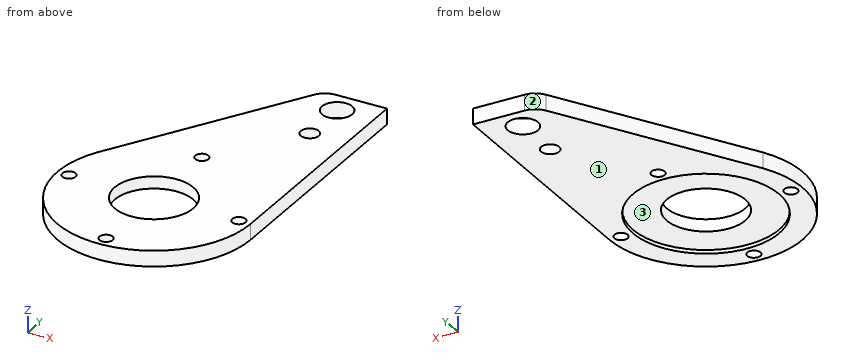
from build123d import *

# Parameters (mm, degrees)
SKETCH_1_R          = 32.5
SKETCH_1_R_2        = 12.5
SKETCH_1_R_3        = 7.5
EXTRUDE_1_DEPTH     = 13
CUT_EXTRUDE_START   = 3
SKETCH_2_R          = 60.5
CUT_EXTRUDE_2_DEPTH = 219.79851714
SKETCH_4_R          = 5.5
CUT_EXTRUDE_3_DEPTH = 216.79851714


with BuildPart() as part:
    # 草图1 → 凸台-拉伸1 (new body)
    with BuildSketch(Plane.XY):
        with BuildLine():
            Line((80, 200), (37.5, 200))
            ThreePointArc((37.5, 200), (29.674290769, 197.955582218), (23.848458927, 192.34478438))
            Line((23.848458927, 192.34478438), (-69.388730207, 39.814621941))
            ThreePointArc((-69.388730207, 39.814621941), (-20.602203565, -77.30167662), (80, 0))
            Line((80, 0), (80, 160))
            Line((80, 160), (80, 200))
        make_face()
        with Locations(Location((0, 0, 0), (0, 0, 180))):
            Circle(SKETCH_1_R, mode=Mode.SUBTRACT)
        with Locations(Location((50, 180, 0), (0, 0, 180))):
            Circle(SKETCH_1_R_2, mode=Mode.SUBTRACT)
        with Locations(Location((50, 140, 0), (0, 0, 180))):
            Circle(SKETCH_1_R_3, mode=Mode.SUBTRACT)
    extrude(amount=EXTRUDE_1_DEPTH)

    # 草图2 → 切除-拉伸2 (cut, through all)
    with BuildSketch(Plane.XY.offset(CUT_EXTRUDE_START)):
        Circle(SKETCH_2_R)
    extrude(amount=-CUT_EXTRUDE_2_DEPTH, mode=Mode.SUBTRACT)

    # 草图4 → 切除-拉伸3 (cut, through all)
    with BuildSketch(Plane(origin=(0, 0, 0), x_dir=(-1, 0, 0), z_dir=(0, 0, -1))):
        with Locations((70.25, 0)):
            Circle(SKETCH_4_R)
        with Locations((0, -70.25)):
            Circle(SKETCH_4_R)
        with Locations((-70.25, 0)):
            Circle(SKETCH_4_R)
        with Locations((0, 70.25)):
            Circle(SKETCH_4_R)
    extrude(amount=-CUT_EXTRUDE_3_DEPTH, mode=Mode.SUBTRACT)


solid = part.part
Work out the finished part from the listing and answer in its coordinate system (mm). Face numbers are marked on the shaded views. Round coordinates to 2 decimals unless told otherwise and drop trailing zeros. Write each loop counter-clockwise with the first axis right and the second up, starting at its lowest first coordinate (ties: lowest second). Pieces come first, ordered by that corner, then holes. Notation, with made-up numbers: M 65.5,-6.5 L 120.5,-6.5 A16 ccw 120.5,23.5 Z; hole C 29,27.5 d7. An arc over 180 degrees is marked long. Use a Markdown table: item, result.
1) The part is cut by section A-A on y = -70.25. Give the vertices of the cut face in (x, z), plus the area to 3 significant figures.
Taken from the geometry:
| item | result |
|---|---|
| outline | M -38.27,0 L -5.5,0 L -5.5,13 L -38.27,13 Z; M 5.5,0 L 38.27,0 L 38.27,13 L 5.5,13 Z |
| area | 852 mm2 |
2) Determine the mould class of the marked faces 1, 2 and 3 for opening direction Y: pulls with the +Y half, pulls with the -Y half, needs draft (parallel to the pull), parting line crosses it, or undercut.
Taken from the geometry:
| item | result |
|---|---|
| face 1 | needs draft |
| face 2 | pulls with the +Y half |
| face 3 | undercut |
3) Flat-ended cylindrical pins translate along their axes: pin 1 (1.5 mm diameter, centred on x = 9, z = 7.5, fed in from -Y); pin 2 (2 mm diameter, centred on x = -19, z = 1.5, fed in from -Y); pin 3 (1 mm diameter, centred on y = 160, z = 10, fed in from -X). Find the tip coordinate at first contact, or state that the pin passes through.
Taken from the geometry:
| item | result |
|---|---|
| pin 1 | stops at y = -79.57 |
| pin 2 | stops at y = -77.95 |
| pin 3 | stops at x = 3.77 |
4) The part is cut by section B-B on x = 54. Give the vertices of the cut face in (y, z).
Taken from the geometry:
| item | result |
|---|---|
| outline | M -59.03,0 L -27.28,0 L -27.28,3 L 27.28,3 L 27.28,0 L 133.66,0 L 133.66,13 L -59.03,13 Z; M 146.34,0 L 168.16,0 L 168.16,13 L 146.34,13 Z; M 191.84,0 L 200,0 L 200,13 L 191.84,13 Z |
5) The part is cut by section D-D on x = 17.5. Give the vertices of the cut face in (y, z).
Taken from the geometry:
| item | result |
|---|---|
| outline | M -78.06,0 L -57.91,0 L -57.91,3 L -27.39,3 L -27.39,13 L -78.06,13 Z; M 27.39,3 L 57.91,3 L 57.91,0 L 181.96,0 L 181.96,13 L 27.39,13 Z |
6) The part is cut by section C-C on z = 8. Give the vertices of the cut face in (x, y), plus the area to 3 significant figures.
Taken from the geometry:
| item | result |
|---|---|
| outline | M -69.39,39.81 A80 ccw long 80,0 L 80,200 L 37.5,200 A16 ccw 23.85,192.34 Z; hole C -70.25,0 d11; hole C 0,0 d65; hole C 0,-70.25 d11; hole C 0,70.25 d11; hole C 50,180 d25; hole C 50,140 d15; hole C 70.25,0 d11 |
| area | 28,000 mm2 |
7) Consider line 1 (Y direction, x = 50, z = 6.5); line 2 (Y direction, x = 52.5, z = 5.25); line 3 (Z direction, x = 38, y = -28). Determine where each line is inside the solid, lowest interval first. Write a range as [from, to].
Taken from the geometry:
| item | result |
|---|---|
| line 1 | y = [-62.45, 132.5], [147.5, 167.5], [192.5, 200] |
| line 2 | y = [-60.36, 132.93], [147.07, 167.75], [192.25, 200] |
| line 3 | z = [3, 13] |
